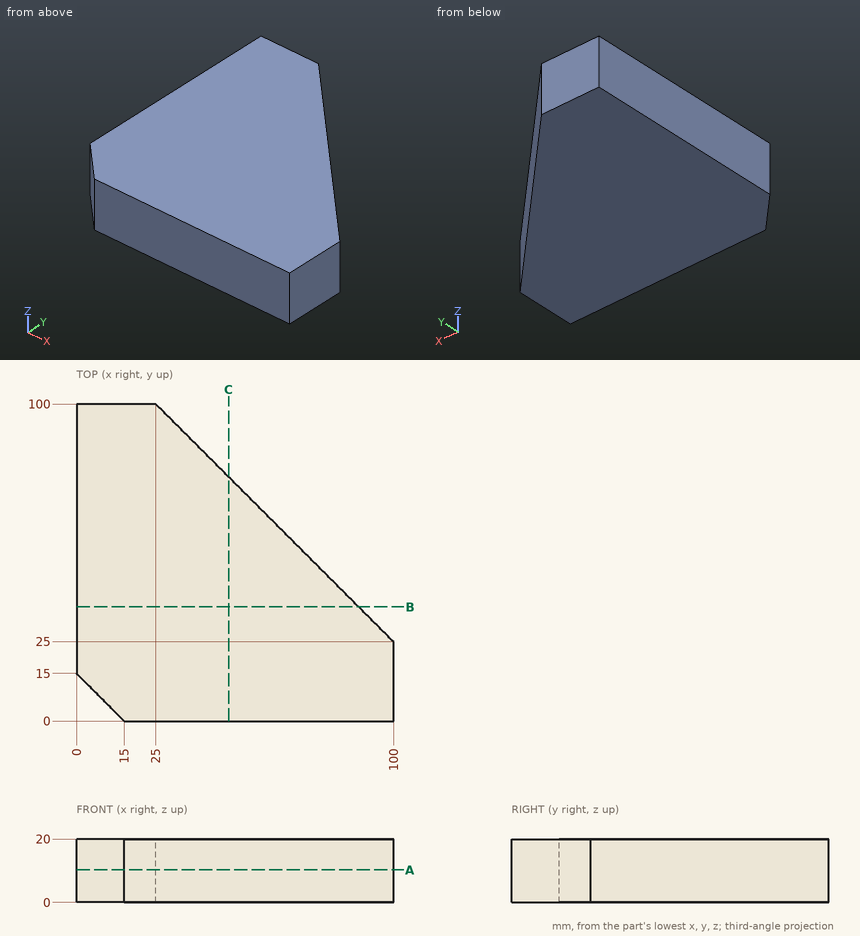
Input: dimensioned drawing with shaded views. Units: mm. Origin: part minimum x, y, z. Coordinates: 2 decimals unless noted, no trailing zeros. Order: outer loops, then holes, each group sorted by start corner. A loop starts at its lowest first (then second) coordinate and runs counter-clockwise, first axis right, second up.
(1) Material intervals for probe 1 along X at (y, z) = (34, 8.5); probe 2 along X at (y, z) = (38.5, 11.75); probe 3 along Y at (x, z) = (90, 4.25), sorted ascending.
(2) First-contact query: pin 1 (5 mm diameter, centred on x = 47, z = 6.5, fed in from +Y); pin 2 (2 mm diameter, centred on x = 48, y = 75, fed in from -Z); pin 3 (1.5 mm diameter, centred on x = 50.5, z = 16.5, fed in from +Y); pin 4 (1.5 mm diameter, centred on y = 42, z = 3, fed in from +X). Flat tips, straight axial feed; report the tip coordinate or a pass-through.
(3) Section query B-B (y = 36). Return the cut outline in (x, z), plus the area to 3 significant figures.
(4) Section query C-C (x = 48). Return the cut outline in (y, z), plus the area to 3 significant figures.
(5) Section query A-A (z = 10.25). Return the cut outline in (x, y).
Solution:
1. probe 1: x = 0 to 91
1. probe 2: x = 0 to 86.5
1. probe 3: y = 0 to 35
2. pin 1: stops at y = 80.5
2. pin 2: stops at z = 0
2. pin 3: stops at y = 75.25
2. pin 4: stops at x = 83.75
3. outline: (0, 0) - (89, 0) - (89, 20) - (0, 20) - close
3. area: 1,780 mm2
4. outline: (0, 0) - (77, 0) - (77, 20) - (0, 20) - close
4. area: 1,540 mm2
5. outline: (0, 15) - (15, 0) - (100, 0) - (100, 25) - (25, 100) - (0, 100) - close
